Design review of the part shown in the three views and the two pictorial views. Dimensions are in mm from the part's minimum x, y and z. Give positions to 0.01 mm unless a question says otherwise; leave off trailing zeros. Order: outer loops, then holes, each group sorted by start corner. A loop starts at its lowest first (then second) coordinate and runs counter-clockwise, first axis right, second up.
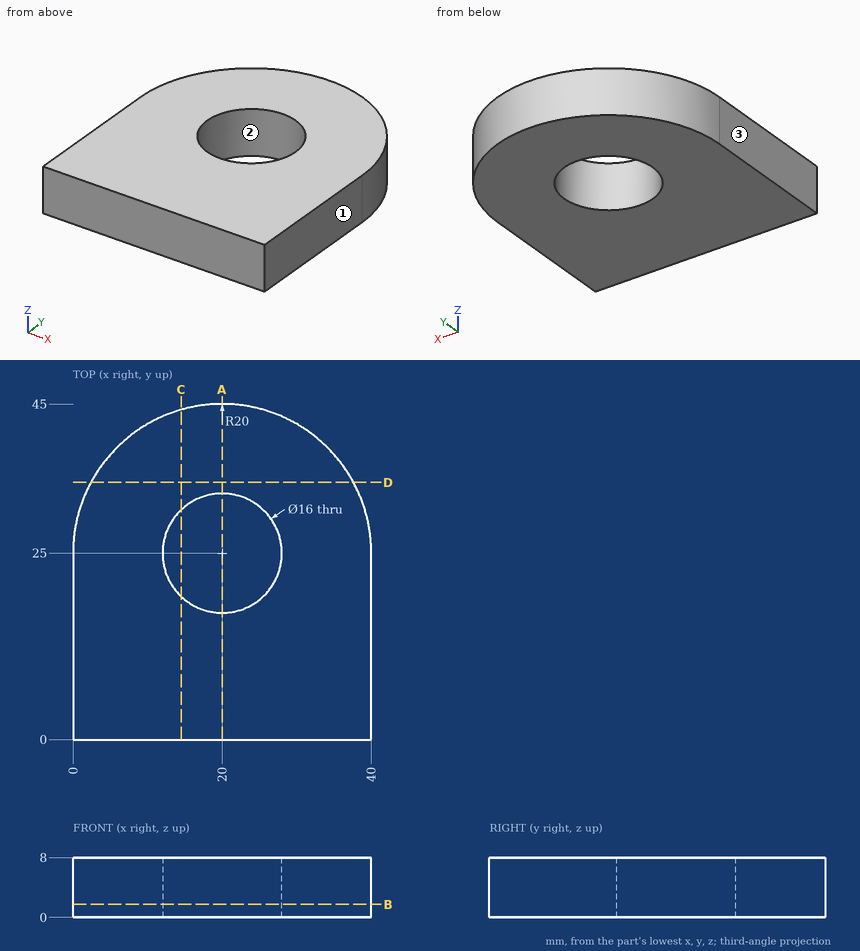
1) Clearance check with flat-ended pins moving along their axes: pin 1 (5 mm diameter, centred on x = 23, y = 20.5, fed in from -Z); pin 2 (3 mm diameter, centred on x = 20, z = 3.5, fed in from +Y). State where each tip first meets the part, or that it passes through.
Answer sheet:
pin 1: passes through
pin 2: stops at y = 45
2) We need section D-D on y = 34.5. Give the boundary of the cut face in (x, z), then the cut area to 3 significant figures.
Answer sheet:
outline: (2.4, 0) - (37.6, 0) - (37.6, 8) - (2.4, 8) - close
area: 282 mm2
3) Draft analysis for pull direction X (two halves, no side actions). For the marked faces 1, 2 and 3, state which applies: +X half, -X half, draft (parallel to the pull), parting line (faces both ways), or undercut.
Answer sheet:
face 1: +X half
face 2: undercut
face 3: -X half
4) We need section B-B on z = 1.75. Give the boundary of the cut face in (x, y), then the cut area to 3 significant figures.
Answer sheet:
outline: (0, 0) - (40, 0) - (40, 25) arc R20 ccw to (0, 25) - close; hole circle Ø16 at (20, 25)
area: 1,430 mm2
5) To check wall thickness, follow line 1 (Y direction, x = 20, z = 6); line 2 (X direction, y = 29, z = 3.25); line 3 (X direction, y = 22, z = 7). State the ranges of each line that lie inside material, in increasing order.
Answer sheet:
line 1: y = 0 to 17, 33 to 45
line 2: x = 0.4 to 13.07, 26.93 to 39.6
line 3: x = 0 to 12.58, 27.42 to 40
6) We need section C-C on x = 14.5. Give the boundary of the cut face in (y, z).
Answer sheet:
outline: (0, 0) - (19.19, 0) - (19.19, 8) - (0, 8) - close; (30.81, 0) - (44.23, 0) - (44.23, 8) - (30.81, 8) - close
7) We need section A-A on x = 20. Give the boundary of the cut face in (y, z).
Answer sheet:
outline: (0, 0) - (17, 0) - (17, 8) - (0, 8) - close; (33, 0) - (45, 0) - (45, 8) - (33, 8) - close
